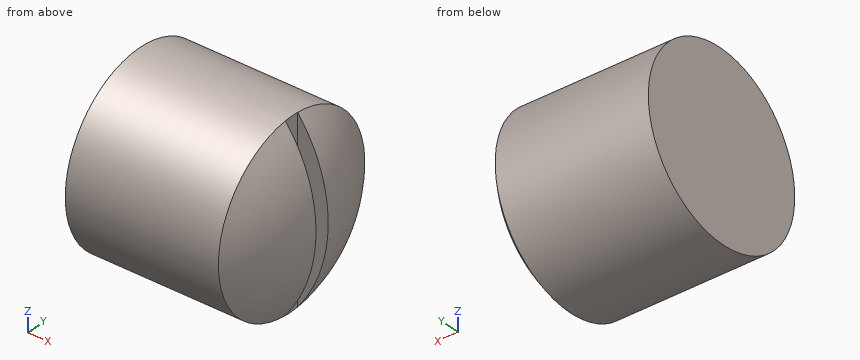
```python
from build123d import *

# Parameters (mm, degrees)
CUT_EXTRUDE1_DEPTH      = 30.393876913
CUT_EXTRUDE1_DEPTH_BACK = 30.393876913
SKETCH2_W               = 8
SKETCH2_H               = 2


with BuildPart() as part:
    # Sketch1 → Revolve1 (revolve)
    with BuildSketch(Plane.XY, mode=Mode.PRIVATE) as revolve1_sk:
        with BuildLine():
            Line((0, 0), (0, 12))
            Line((0, 12), (20, 12))
            ThreePointArc((20, 12), (22.973665961, 6.32455532), (24, 0))
            Line((24, 0), (0, 0))
        make_face()
    revolve(revolve1_sk.sketch.rotate(Axis((0, 0, 0), (1, 0, 0)), 90), axis=Axis((0, 0, 0), (1, 0, 0)))

    # Sketch2 → Cut-Extrude1 (cut, two sides: drawn at the far end of the back side and taken through both)
    with BuildSketch(Plane.XY.offset(-CUT_EXTRUDE1_DEPTH_BACK)):
        with Locations((24, 0)):
            Rectangle(SKETCH2_W, SKETCH2_H)
    extrude(amount=CUT_EXTRUDE1_DEPTH + CUT_EXTRUDE1_DEPTH_BACK, mode=Mode.SUBTRACT)


solid = part.part
```
Geometry check sheet. Reference: the model listing, model coordinates, mm. Round coordinates to 2 decimals unless told otherwise and drop trailing zeros. Loops run counter-clockwise (first coordinate to the right, second up) from the corner with the lowest first, then second, coordinate; pieces in that order, holes last. Notation, with made-up numbers: (85.25, 48.5) - (138.25, 48.5) arc R18 cw to (138.25, 61.5) - close; hole circle Ø10 at (34, 15). An arc over 180 degrees is marked (long way). Write item = value, one per line. Start each with the question number.
1. Section check D-D on x = 16.5. Enter the section's corners in (y, z), then the cut area to 3 significant figures.
2. Thickness scan on line 1 (Z direction, x = 15.5, y = -0.25); line 2 (Y direction, x = 19.25, z = -7.25); line 3 (Z direction, x = 15.75, y = 6.5). Record the ranges inside material, lowest first.
3. Section check C-C on x = 22.5. Enter the section's corners in (y, z).
4. Depth check by flat-ended pin: pin 1 (8 mm diameter, centred on x = 8.5, y = -5, fed in from +Z); pin 2 (3 mm diameter, centred on x = 6, y = 8, fed in from +Z); pin 3 (6 mm diameter, centred on y = 3, z = 5.5, fed in from -X); pin 4 (1 mm diameter, centred on x = 10.5, y = 6.5, fed in from +Z). Enter the tip coordinate at first touch or a pass-through.
5. Section check B-B on y = -10.25. Enter the section's corners in (x, z).
6. Section check A-A on z = 0. Enter the section's corners in (x, y).
Working result:
q1.outline = circle Ø24 at (0, 0)
q1.area = 452 mm^2
q2.line_1 = -12 to 12
q2.line_2 = -9.56 to 9.56
q2.line_3 = -10.09 to 10.09
q3.outline = (-1, -7.53) - (-1, 7.53) arc R7.6 ccw to start; (1, -7.53) arc R7.6 ccw to (1, 7.53) - close
q4.pin_1 = 11.96
q4.pin_2 = 10.09
q4.pin_3 = 0
q4.pin_4 = 10.39
q5.outline = (0, -6.24) - (20, -6.24) arc R17.17 ccw to (20, 6.24) - (0, 6.24) - close
q6.outline = (0, -12) - (20, -12) arc R20 ccw to (23.97, -1) - (20, -1) - (20, 1) - (23.97, 1) arc R20 ccw to (20, 12) - (0, 12) - close
